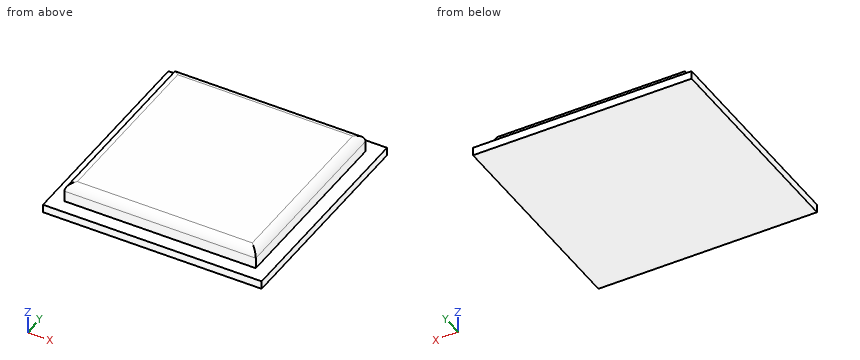
from build123d import *

# Parameters (mm, degrees)
SKETCH1_W           = 80
SKETCH1_H           = 80
BOSS_EXTRUDE1_DEPTH = 3
SKETCH2_W           = 70
SKETCH2_H           = 70
BOSS_EXTRUDE2_DEPTH = 7
FILLET1_R           = 3


with BuildPart() as part:
    # Sketch1 → Boss-Extrude1 (new body)
    with BuildSketch(Plane.XY):
        Rectangle(SKETCH1_W, SKETCH1_H)
    extrude(amount=BOSS_EXTRUDE1_DEPTH)

    # Sketch2 → Boss-Extrude2 (add)
    with BuildSketch(Plane.XY.offset(3)):
        Rectangle(SKETCH2_W, SKETCH2_H)
    extrude(amount=BOSS_EXTRUDE2_DEPTH)

    # Fillet1
    fillet1_edges = [part.edges().sort_by_distance(p)[0] for p in [
        (35, 0, 10),
        (0, 35, 10),
        (-35, 0, 10),
        (0, -35, 10),
    ]]
    fillet(fillet1_edges, radius=FILLET1_R)


solid = part.part
For this review, take the finished solid that the model builds, in its own axes (mm). Round coordinates to 2 decimals unless told otherwise and drop trailing zeros. Order: outer loops, then holes, each group sorted by start corner. A loop starts at its lowest first (then second) coordinate and runs counter-clockwise, first axis right, second up. Notation, with made-up numbers: M 6.5,51.25 L 13.5,51.25 A12 ccw 13.5,58.25 Z; hole C 16.5,77 d3. An arc over 180 degrees is marked long. Use a Markdown table: item, result. Add a question column.
Item 1: Add section C-C, the plane z = 4.25. Give the boundary of the cut face in (x, y).
Item 2: Insertion check: pin 1 (2 mm diameter, centred on y = -0.5, z = 5, fed in from +X). The pin has a flat end and moves straight along its axis. Give the tip position at first contact, or say it passes through.
Item 3: Add section A-A, the plane y = 18. Give the boundary of the cut face in (x, z).
Item 4: To check wall thickness, follow line 1 along X through (y, z) = (30, 5.75); line 2 along Z through (x, y) = (-36, -23.5). State the ranges of each line that lie inside material, in increasing order.
Item 5: Add section D-D, the plane z = 8.25. Give the boundary of the cut face in (x, y).
Geometry results:
| question | item | result |
|---|---|---|
| 1 | outline | M -35,-35 L 35,-35 L 35,35 L -35,35 Z |
| 2 | pin 1 | stops at x = 35 |
| 3 | outline | M -40,0 L 40,0 L 40,3 L 35,3 L 35,7 A3 ccw 32,10 L -32,10 A3 ccw -35,7 L -35,3 L -40,3 Z |
| 4 | line 1 | x = -35 to 35 |
| 4 | line 2 | z = 0 to 3 |
| 5 | outline | M -34.73,-34.73 L 34.73,-34.73 L 34.73,34.73 L -34.73,34.73 Z |
